Could you check a few things on this model? Use its own coordinates, in mm. A direction names the side the tool comes from. Give positions to 0.01 mm unless a question says otherwise; leave off trailing zeros. Loops run counter-clockwise (first coordinate to the right, second up) from the corner with the lowest first, then second, coordinate; pieces in that order, holes last. Notation, with made-up numbers: (9, -28.5) -> (45, -28.5) arc R22 ccw to (45, -2.5) -> close; hole circle Ø9 at (46, 18). An arc over 180 degrees is marked (long way). Put each result on its own line as item: value.
```python
from build123d import *

# Parameters (mm, degrees)
SKETCH1_R           = 185
SKETCH1_R_2         = 101
BOSS_EXTRUDE1_DEPTH = 12
SKETCH2_R           = 129.75
CUT_EXTRUDE1_DEPTH  = 4
BOSS_EXTRUDE2_START = 4
SKETCH3_R           = 134.75
SKETCH3_R_2         = 129.75
BOSS_EXTRUDE2_DEPTH = 4
SKETCH4_R           = 7
CUT_EXTRUDE2_DEPTH  = 262.90456277
CIRPATTERN1_COUNT   = 6


with BuildPart() as part:
    # Sketch1 → Boss-Extrude1 (new body)
    with BuildSketch(Plane(origin=(0, 0, 0), x_dir=(1, 0, 0), z_dir=(0, 1, 0))):
        with Locations(Location((0, 0, 0), (0, 0, 270))):
            Circle(SKETCH1_R)
        with Locations(Location((0, 0, 0), (0, 0, 270))):
            Circle(SKETCH1_R_2, mode=Mode.SUBTRACT)
    extrude(amount=BOSS_EXTRUDE1_DEPTH)

    # Sketch2 → Cut-Extrude1 (cut)
    with BuildSketch(Plane(origin=(0, 12, 0), x_dir=(1, 0, 0), z_dir=(0, 1, 0))):
        with Locations(Location((0, 0, 0), (0, 0, 270))):
            Circle(SKETCH2_R)
    extrude(amount=-CUT_EXTRUDE1_DEPTH, mode=Mode.SUBTRACT)

    # Sketch3 → Boss-Extrude2 (add)
    with BuildSketch(Plane(origin=(0, 12, 0), x_dir=(1, 0, 0), z_dir=(0, 1, 0)).offset(BOSS_EXTRUDE2_START)):
        with Locations(Location((0, 0, 0), (0, 0, 270))):
            Circle(SKETCH3_R)
        with Locations(Location((0, 0, 0), (0, 0, 270))):
            Circle(SKETCH3_R_2, mode=Mode.SUBTRACT)
    extrude(amount=-BOSS_EXTRUDE2_DEPTH)

    # Sketch4 → Cut-Extrude2 (cut, through all)
    with BuildSketch(Plane(origin=(0, 12, 0), x_dir=(1, 0, 0), z_dir=(0, 1, 0))):
        with Locations(Location((160, 0, 0), (0, 0, 270))):
            Circle(SKETCH4_R)
    cut_extrude2 = extrude(amount=-CUT_EXTRUDE2_DEPTH, mode=Mode.SUBTRACT)

    # CirPattern1: Cut-Extrude2 ×6 about axis
    cirpattern1_axis = Axis((0, 0, 0), (0, 1, 0))
    for i in range(1, CIRPATTERN1_COUNT):
        add(cut_extrude2.rotate(cirpattern1_axis, i * 360 / CIRPATTERN1_COUNT), mode=Mode.SUBTRACT)


solid = part.part
```
1. If we section it at D-D (z = -85): List the corners of the cut face in (x, y) for me, then the cut area to 3 significant figures.
Recorded:
outline: (-164.32, 0) -> (-54.55, 0) -> (-54.55, 8) -> (-98.03, 8) -> (-98.03, 16) -> (-104.56, 16) -> (-104.56, 12) -> (-164.32, 12) -> close; (54.55, 0) -> (164.32, 0) -> (164.32, 12) -> (104.56, 12) -> (104.56, 16) -> (98.03, 16) -> (98.03, 8) -> (54.55, 8) -> close
area: 2,340 mm^2
2. I need wall thicknesses on line 1 (X direction, y = 8.75, z = 0); line 2 (X direction, y = 6, z = 0); line 3 (X direction, y = 3.5, z = -136). Which ranges of each line are inside material? Lowest first, please.
Recorded:
line 1: x = -185 to -167, -153 to -129.75, 129.75 to 153, 167 to 185
line 2: x = -185 to -167, -153 to -101, 101 to 153, 167 to 185
line 3: x = -125.42 to -86.51, -73.49 to 73.49, 86.51 to 125.42
3. I'm going to push flat-ended pins straight in: pin 1 (1.5 mm diameter, centred on y = 4, z = 121, fed in from +X); pin 2 (3 mm diameter, centred on y = 8, z = -34.5, fed in from -X); pin 3 (22.5 mm diameter, centred on x = -160, z = 0, fed in from +Y); pin 4 (11 mm diameter, centred on x = -80, z = -138.56, fed in from -Y). Where does each tip first touch, or does it pass through?
Recorded:
pin 1: stops at x = 140.59
pin 2: stops at x = -182.03
pin 3: stops at y = 12
pin 4: passes through
4. Thinking about a two-plate mould opening in X: for faces 1 (the face through (-131.546, 14.028, -29.211)), 2 (the face through (-109, 12, -83)), 3 (the face through (-84.26, 6.08, 133.01)), which applies, pulls with the +X half, pulls with the -X half, needs draft (parallel to the pull), parting line crosses it, or undercut?
Recorded:
face 1: parting line crosses it
face 2: needs draft
face 3: undercut
5. If we section it at B-B (z = 0): List the corners of the cut face in (x, y) for me.
Recorded:
outline: (-185, 0) -> (-167, 0) -> (-167, 12) -> (-185, 12) -> close; (-153, 0) -> (-101, 0) -> (-101, 8) -> (-129.75, 8) -> (-129.75, 16) -> (-134.75, 16) -> (-134.75, 12) -> (-153, 12) -> close; (101, 0) -> (153, 0) -> (153, 12) -> (134.75, 12) -> (134.75, 16) -> (129.75, 16) -> (129.75, 8) -> (101, 8) -> close; (167, 0) -> (185, 0) -> (185, 12) -> (167, 12) -> close
6. If we section it at A-A (x = 0): List the corners of the cut face in (y, z) for me.
Recorded:
outline: (0, -185) -> (12, -185) -> (12, -134.75) -> (16, -134.75) -> (16, -129.75) -> (8, -129.75) -> (8, -101) -> (0, -101) -> close; (0, 101) -> (8, 101) -> (8, 129.75) -> (16, 129.75) -> (16, 134.75) -> (12, 134.75) -> (12, 185) -> (0, 185) -> close
7. For faces 4 (the face through (-61.46, 3.94, -80.15)), 5 (the face through (38.97, 12.06, 123.76)), which set-ups out of +Z, -Z, +X, -X, +Y, -Y let a thin tool reach every point of the face, with its end or its side?
Recorded:
face 4: +Y, -Y
face 5: +Y
8. If we section it at C-C (y = 3.5): List the corners of the cut face in (x, z) for me.
Recorded:
outline: circle Ø370 at (0, 0); hole circle Ø14 at (-160, 0); hole circle Ø202 at (0, 0); hole circle Ø14 at (-80, -138.56); hole circle Ø14 at (-80, 138.56); hole circle Ø14 at (80, -138.56); hole circle Ø14 at (80, 138.56); hole circle Ø14 at (160, 0)
